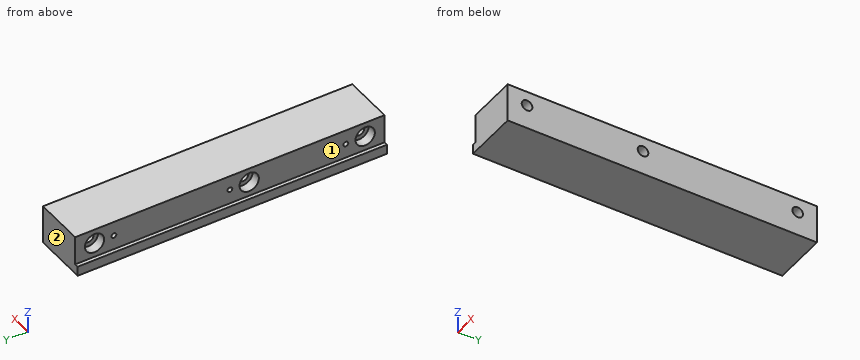
from build123d import *

# Parameters (mm, degrees)
SKETCH_1_W                                         = 20
SKETCH_1_H                                         = 160
BOSS_EXTRUDE_1_DEPTH                               = 28
SKETCH_2_W                                         = 15
SKETCH_2_H                                         = 160
CUT_EXTRUDE_1_DEPTH                                = 2
LINEAR_PATTERN_1_COUNT                             = 3
LINEAR_PATTERN_1_PITCH                             = 60
M5_SOCKET_HEAD_CAP_SCREW_COUNTERBORE_1_D           = 5.5
M5_SOCKET_HEAD_CAP_SCREW_COUNTERBORE_1_CBORE_D     = 10
M5_SOCKET_HEAD_CAP_SCREW_COUNTERBORE_1_CBORE_DEPTH = 5
LINEAR_PATTERN_2_COUNT                             = 2
LINEAR_PATTERN_2_PITCH                             = 140
LINEAR_PATTERN_3_COUNT                             = 2
LINEAR_PATTERN_3_PITCH                             = 60


with BuildPart() as part:
    # Sketch 1 → Boss-Extrude 1 (new body)
    with BuildSketch(Plane(origin=(0, 0, 0), x_dir=(0, 0, -1), z_dir=(1, 0, 0))):
        Rectangle(SKETCH_1_W, SKETCH_1_H)
    extrude(amount=BOSS_EXTRUDE_1_DEPTH)

    # Sketch 2 → Cut-Extrude 1 (cut)
    with BuildSketch(Plane.ZY):
        with Locations((2.5, 0)):
            Rectangle(SKETCH_2_W, SKETCH_2_H)
    extrude(amount=-CUT_EXTRUDE_1_DEPTH, mode=Mode.SUBTRACT)

    # Sketch 3 → M3 Tapped Hole 1 (revolve, cut)
    with BuildSketch(Plane(origin=(2, -60, 2.5), x_dir=(0, 0, 1), z_dir=(0, 1, 0))):
        Polygon((0, 0), (0, 8.251075774), (1.25, 7.5), (1.25, 0), align=None)
    m3_tapped_hole_1 = revolve(axis=Axis((-4.35, -60, 2.5), (1, 0, 0)), mode=Mode.SUBTRACT)

    # Linear Pattern 1: M3 Tapped Hole 1 ×3
    with Locations(*[(0, i * LINEAR_PATTERN_1_PITCH, 0) for i in range(1, LINEAR_PATTERN_1_COUNT)]):
        add(m3_tapped_hole_1, mode=Mode.SUBTRACT)

    # M5 Socket Head Cap Screw Counterbore 1 (through all)
    with Locations(Plane.ZY.offset(-2)):
        with Locations((2.5, -70)):
            m5_socket_head_cap_screw_counterbore_1 = CounterBoreHole(M5_SOCKET_HEAD_CAP_SCREW_COUNTERBORE_1_D / 2, M5_SOCKET_HEAD_CAP_SCREW_COUNTERBORE_1_CBORE_D / 2, M5_SOCKET_HEAD_CAP_SCREW_COUNTERBORE_1_CBORE_DEPTH)

    # Linear Pattern 2: M5 Socket Head Cap Screw Counterbore 1 ×2
    with Locations(*[(0, i * LINEAR_PATTERN_2_PITCH, 0) for i in range(1, LINEAR_PATTERN_2_COUNT)]):
        add(m5_socket_head_cap_screw_counterbore_1, mode=Mode.SUBTRACT)

    # Linear Pattern 3: M5 Socket Head Cap Screw Counterbore 1 ×2
    with Locations(*[(0, i * LINEAR_PATTERN_3_PITCH, 0) for i in range(1, LINEAR_PATTERN_3_COUNT)]):
        add(m5_socket_head_cap_screw_counterbore_1, mode=Mode.SUBTRACT)


solid = part.part
Here's how the part is built. I have some questions about the finished solid (model axes, mm). Face numbers are marked on the shaded views. A direction names the side the tool comes from. Coordinates: 2 decimals unless noted, no trailing zeros. Loops run counter-clockwise (first coordinate to the right, second up) from the corner with the lowest first, then second, coordinate; pieces in that order, holes last.
1. I need wall thicknesses on L1, parallel to Y at x = 22.75, z = 2.5; L2, parallel to Y at x = 9, z = 0; L3, parallel to X at y = -23.5, z = 7. Which ranges of each line are inside material? Lowest first, please.
2. For the marked faces 1 and 2, which set-ups out of +Z, -Z, +X, -X, +Y, -Y let a thin tool reach every point of the face, with its end or its side?
3. Imagine slicing it at A-A, the plane y = 70. Please give me the cut outline in (x, z), and give its area (4 significant figures).
4. Imagine slicing it at B-B, the plane x = 18. Please give me the cut outline in (y, z), and give its area (3 significant figures).
5. For P1, Ø6.5, axis at y = -70, z = 2.5, coming from the -X side; P2, Ø8, axis at y = 69.5, z = 1.5, coming from the -X side; P3, Ø2, axis at y = 0, z = 2.5, coming from the -X side, each with a flat end and sliding along its axis, tell me the tip position at first contact or that it passes through.
6. Imagine slicing it at C-C, the plane y = 5.5. Please give me the cut outline in (x, z).
Taken from the geometry:
1. L1: y = -80 to -72.75, -67.25 to -12.75, -7.25 to 67.25, 72.75 to 80
1. L2: y = -80 to -71.15, -68.85 to -11.15, -8.85 to 68.85, 71.15 to 80
1. L3: x = 2 to 28
2. face 1: +Z, -X, +Y, -Y
2. face 2: +Z, -Z, +X, -X, +Y
3. outline: (0, -10) - (28, -10) - (28, -0.25) - (7, -0.25) - (7, -2.5) - (2, -2.5) - (2, -5) - (0, -5) - close; (2, 7.5) - (7, 7.5) - (7, 5.25) - (28, 5.25) - (28, 10) - (2, 10) - close
3. area: 364.5 mm2
4. outline: (-80, -10) - (80, -10) - (80, 10) - (-80, 10) - close; hole circle Ø5.5 at (-70, 2.5); hole circle Ø5.5 at (-10, 2.5); hole circle Ø5.5 at (70, 2.5)
4. area: 3,130 mm2
5. P1: stops at x = 7
5. P2: stops at x = 2
5. P3: stops at x = 9.65
6. outline: (0, -10) - (28, -10) - (28, 10) - (2, 10) - (2, -5) - (0, -5) - close
